Verification items for the finished model (mm, model axes). Give positions to 0.01 mm unless a question says otherwise; leave off trailing zeros. Write each loop counter-clockwise with the first axis right and the second up, starting at its lowest first coordinate (ties: lowest second). Pieces come first, ordered by that corner, then holes. Notation, with made-up numbers: (-1, 55) - (31, 55) arc R19 ccw to (31, 70) - close; hole circle Ø6 at (58.25, 10.25). An arc over 180 degrees is marked (long way). Answer as a JSON object with one key per item and string values. Group by question number.
Item 1: Scan lines: line 1 along X through (y, z) = (9, 2.75); line 2 along Y through (x, z) = (-18.5, 2.1); line 3 along Y through (x, z) = (14, 2.15). Record each from-to range of solid material in increasing order. Write a range as [from, to].
Item 2: Sectioned sample at A-A, the plane z = 0.5. Record the boundary of the cut face in (x, y).
Item 3: Sectioned sample at D-D, the plane y = 4. Record the boundary of the cut face in (x, z), and give its area (4 significant figures).
Item 4: Draft check along X on faces 1 (the face through (1.28, -3.79, 2.46)), 2 (the face through (0, -2, 2)), 3 (the face through (-3, 8, 5)). Enter one of: +X half, -X half, draft (parallel to the pull), parting line (faces both ways), or undercut.
Item 5: Sectioned sample at C-C, the plane x = -16. Record the boundary of the cut face in (y, z).
Item 6: Sectioned sample at B-B, the plane y = 0. Record the boundary of the cut face in (x, z).
```python
from build123d import *

# Parameters (mm, degrees)
SKETCH1_R           = 2
SKETCH1_R_2         = 3
BOSS_EXTRUDE1_DEPTH = 5


with BuildPart() as part:
    # Sketch1 → Boss-Extrude1 (new body)
    with BuildSketch(Plane.XY):
        with BuildLine():
            Line((-17.245659368, 15.645832119), (12.135648337, 20.594443797))
            ThreePointArc((12.135648337, 20.594443797), (16.228516711, 18.710406067), (15.971203863, 14.212077511))
            Line((15.971203863, 14.212077511), (3.171203863, -2.437922489))
            ThreePointArc((3.171203863, -2.437922489), (1.248757853, -3.80007945), (-1.106950177, -3.843782162))
            Line((-1.106950177, -3.843782162), (-18.075531582, 1.042908447))
            ThreePointArc((-18.075531582, 1.042908447), (-23.487918421, 8.675532282), (-17.245659368, 15.645832119))
        make_face()
        Circle(SKETCH1_R, mode=Mode.SUBTRACT)
        with Locations((-16, 8.25)):
            Circle(SKETCH1_R_2, mode=Mode.SUBTRACT)
        with Locations((12.8, 16.65)):
            Circle(SKETCH1_R, mode=Mode.SUBTRACT)
    extrude(amount=BOSS_EXTRUDE1_DEPTH)


solid = part.part
```
Geometry check:
{
 "1": {"line 1": "[-23.46, -18.9], [-13.1, 11.96]", "line 2": "[1.18, 6.59], [9.91, 15.32]", "line 3": "[11.65, 15.05], [18.25, 20.47]"},
 "2": {"outline": "(-18.08, 1.04) - (-1.11, -3.84) arc R4 ccw to (3.17, -2.44) - (15.97, 14.21) arc R4 ccw to (12.14, 20.59) - (-17.25, 15.65) arc R7.5 ccw to start; hole circle Ø6 at (-16, 8.25); hole circle Ø4 at (0, 0); hole circle Ø4 at (12.8, 16.65)"},
 "3": {"outline": "(-22.18, 0) - (8.12, 0) - (8.12, 5) - (-22.18, 5) - close", "area": "151.5 mm^2"},
 "4": {"face 1": "parting line", "face 2": "undercut", "face 3": "draft"},
 "5": {"outline": "(0.45, 0) - (5.25, 0) - (5.25, 5) - (0.45, 5) - close; (11.25, 0) - (15.86, 0) - (15.86, 5) - (11.25, 5) - close"},
 "6": {"outline": "(-14.45, 0) - (-2, 0) - (-2, 5) - (-14.45, 5) - close; (2, 0) - (5.05, 0) - (5.05, 5) - (2, 5) - close"}
}
